```python
from build123d import *

# Parameters (mm, degrees)
EXTRUDE_1_DEPTH       = 1.5
HOLE_WIZARD_6_0_6_1_D = 6
FILLET_1_R            = 3


with BuildPart() as part:
    # 草图1 → 凸台-拉伸1 (new body)
    with BuildSketch(Plane.XY):
        Polygon((-12.5, 0), (12.5, 0), (12.5, -15), (0, -27.5), (-12.5, -15), align=None)
    extrude(amount=EXTRUDE_1_DEPTH)

    # Ø6.0 (6) 直径孔1 (through all)
    with Locations(Plane.XY.offset(1.5)):
        with Locations((-7.5, -6), (7.5, -6)):
            Hole(HOLE_WIZARD_6_0_6_1_D / 2)

    # 圆角1
    fillet_1_edges = [part.edges().sort_by_distance(p)[0] for p in [
        (-12.5, 0, 0.75),
        (12.5, 0, 0.75),
    ]]
    fillet(fillet_1_edges, radius=FILLET_1_R)


solid = part.part
```
Here's how the part is built. I have some questions about the finished solid (model axes, mm). Coordinates: 2 decimals unless noted, no trailing zeros. Loops run counter-clockwise (first coordinate to the right, second up) from the corner with the lowest first, then second, coordinate; pieces in that order, holes last. Notation, with made-up numbers: (41.5, -37) -> (72.5, -37) arc R20 cw to (72.5, -4) -> close; hole circle Ø10 at (26, 21.25). An arc over 180 degrees is marked (long way). Return JSON: item names as keys, results as strings.
1) I need wall thicknesses on line 1 (X direction, y = -5, z = 0.65); line 2 (X direction, y = -7.5, z = 0.4); line 3 (Y direction, x = 6.5, z = 1.2). Which ranges of each line are inside material? Lowest first, please. Write a range as from..to.
Results below:
{"line 1": "-12.5..-10.33, -4.67..4.67, 10.33..12.5", "line 2": "-12.5..-10.1, -4.9..4.9, 10.1..12.5", "line 3": "-21..-8.83, -3.17..0"}
2) Will this pin go through, and if not, where does the flat tip stop? pin 1 (9.5 mm diameter, centred on x = -7.5, y = -6, fed in from -Z).
Results below:
{"pin 1": "z = 0"}
3) If we section it at C-C, the plane z = 1.15: Write out the boundary of the cut face in (x, y), then the cut area to 3 significant figures.
Results below:
{"outline": "(-12.5, -15) -> (0, -27.5) -> (12.5, -15) -> (12.5, -3) arc R3 ccw to (9.5, 0) -> (-9.5, 0) arc R3 ccw to (-12.5, -3) -> close; hole circle Ø6 at (-7.5, -6); hole circle Ø6 at (7.5, -6)", "area": "471 mm²"}
4) Thinking about a two-plate mould opening in Y: for faces 1 (the face through (-10.36, -5.1, 0.74)), 2 (the face through (-11.6, -0.86, 0.76)), 3 (the face through (12.5, -9, 1)), which applies, +Y half, -Y half, draft (parallel to the pull), parting line (faces both ways), or undercut?
Results below:
{"face 1": "undercut", "face 2": "+Y half", "face 3": "draft"}
5) If we section it at B-B, the plane y = -6: Write out the boundary of the cut face in (x, z).
Results below:
{"outline": "(-12.5, 0) -> (-10.5, 0) -> (-10.5, 1.5) -> (-12.5, 1.5) -> close; (-4.5, 0) -> (4.5, 0) -> (4.5, 1.5) -> (-4.5, 1.5) -> close; (10.5, 0) -> (12.5, 0) -> (12.5, 1.5) -> (10.5, 1.5) -> close"}
6) If we section it at A-A, the plane x = 7.5: Write out the boundary of the cut face in (y, z).
Results below:
{"outline": "(-20, 0) -> (-9, 0) -> (-9, 1.5) -> (-20, 1.5) -> close; (-3, 0) -> (0, 0) -> (0, 1.5) -> (-3, 1.5) -> close"}
7) If we section it at D-D, the plane x = 1.5: Write out the boundary of the cut face in (y, z).
Results below:
{"outline": "(-26, 0) -> (0, 0) -> (0, 1.5) -> (-26, 1.5) -> close"}
